```python
from build123d import *

# Parameters (mm, degrees)
SKETCH_1_R      = 40
EXTRUDE_1_DEPTH = 30
EXTRUDE_1_TAPER = 34
SKETCH_2_R      = 10
EXTRUDE_2_DEPTH = 125
EXTRUDE_3_DEPTH = 15
SKETCH_4_R      = 40
EXTRUDE_4_DEPTH = 5
EXTRUDE_START   = 40
EXTRUDE_5_DEPTH = 15


with BuildPart() as part:
    # 草图1 → 凸台-拉伸1 (new body)
    with BuildSketch(Plane(origin=(0, 0, 0), x_dir=(1, 0, 0), z_dir=(0, 1, 0))):
        Circle(SKETCH_1_R)
    extrude(amount=EXTRUDE_1_DEPTH, taper=EXTRUDE_1_TAPER)

    # 草图2 → 凸台-拉伸2 (add)
    with BuildSketch(Plane(origin=(0, 30, 0), x_dir=(1, 0, 0), z_dir=(0, 1, 0))):
        with Locations(Location((0, 0, 0), (0, 0, 270))):
            Circle(SKETCH_2_R)
    extrude(amount=EXTRUDE_2_DEPTH)

    # 草图3 → 凸台-拉伸3 (add)
    with BuildSketch(Plane(origin=(0, 30, 0), x_dir=(1, 0, 0), z_dir=(0, 1, 0))):
        Polygon((15, -8.660254038), (15, 8.660254038), (0, 17.320508076), (-15, 8.660254038), (-15, -8.660254038), (0, -17.320508076), align=None)
    extrude(amount=EXTRUDE_3_DEPTH)

    # 草图4 → 凸台-拉伸4 (add)
    with BuildSketch(Plane.XZ):
        with Locations(Location((0, 0, 0), (0, 0, 270))):
            Circle(SKETCH_4_R)
    extrude(amount=EXTRUDE_4_DEPTH)

    # 草图5 → 凸台-拉伸5 (add)
    with BuildSketch(Plane(origin=(0, 45, 0), x_dir=(1, 0, 0), z_dir=(0, 1, 0)).offset(EXTRUDE_START)):
        Polygon((0, -17.320508076), (15, -8.660254038), (15, 8.660254038), (0, 17.320508076), (-15, 8.660254038), (-15, -8.660254038), align=None)
    extrude(amount=EXTRUDE_5_DEPTH)


solid = part.part
```
Read the model definition and answer for the solid it produces. Units are mm, in the model's axes. A direction names the side the tool comes from. Give positions to 0.01 mm unless a question says otherwise; leave off trailing zeros. Order: outer loops, then holes, each group sorted by start corner. A loop starts at its lowest first (then second) coordinate and runs counter-clockwise, first axis right, second up.
(1) For faces 4 (the flat face through (-15, 37, 0)), 5 (the flat face through (7.4, 92.4, 13.05)), 6 (the cylindrical face through (-9.76, 127.12, -2.17)), determine the directions among +Z, -Z, +X, -X, +Y, -Y from which every point of the face is accessible in a straight line to the end or side of a thin tool.
(2) Straight lines are drawn through the part: L1, parallel to Y at x = 10, z = -3; L2, parallel to Y at x = -28.5, z = 26.5; L3, parallel to Y at x = -26, z = 12. For each, find the intervals that lie inside material, in ascending order.
(3) Find section A-A (y = 141). Give the vertices of the cut face in (x, z), plus the area to 3 significant figures.
(4) For a pull along Y with two mould halves and no side action, classify faces 1 (the flat face through (0, 155, 0)), 2 (the flat face through (-6.9, 85, 7.5)), 3 (the flat face through (-7.4, 92.4, -13.05)) as released by +Y, released by -Y, zero draft, split by the parting line, or undercut.
(5) Given pin 1 (12 mm diameter, centred on x = 2.5, y = 29, fed in from +Z); pin 2 (12 mm diameter, centred on y = 131, z = -6, fed in from -X); pin 3 (3 mm diameter, centred on y = 97.5, z = -0.5, fed in from -X), each flat-ended and moving along its own axis, determine where each tip first touches the part or whether it passes through.
Result sheet:
1. face 4: +Z, -Z, -X, +Y
1. face 5: +Z, +X, +Y
1. face 6: +Y
2. L1: y = -5 to 45, 85 to 100
2. L2: y = -5 to 1.61
2. L3: y = -5 to 16.85
3. outline: circle Ø20 at (0, 0)
3. area: 314 mm2
4. face 1: released by +Y
4. face 2: undercut
4. face 3: zero draft
5. pin 1: stops at z = 24.39
5. pin 2: stops at x = -10
5. pin 3: stops at x = -15
